Work out the finished part from the listing and answer in its coordinate system (mm). A direction names the side the tool comes from. Round coordinates to 2 decimals unless told otherwise and drop trailing zeros. Loops run counter-clockwise (first coordinate to the right, second up) from the corner with the lowest first, then second, coordinate; pieces in that order, holes last. Notation, with made-up numbers: (78, 29) -> (95, 29) arc R35 cw to (95, 67) -> close; hole circle Ø8 at (80.25, 32.25). An arc over 180 degrees is marked (long way). Use one line per item in the form item = value.
```python
from build123d import *

# Parameters (mm, degrees)
SKETCH_1_W                 = 410
SKETCH_1_H                 = 110
EXTRUDE_1_DEPTH            = 6
HOLE_WIZARD_3_AT_2_COUNT   = 2
HOLE_WIZARD_3_AT_2_PITCH   = 35
HOLE_WIZARD_3_AT_3_COUNT   = 2
HOLE_WIZARD_3_AT_3_PITCH   = 35
HOLE_WIZARD_3_AT_4_COUNT   = 2
HOLE_WIZARD_3_AT_4_PITCH   = 49.497474683
PATTERN_LINEAR_1_COUNT     = 2
PATTERN_LINEAR_1_PITCH     = 345
HOLE_WIZARD_2_D            = 9
HOLE_WIZARD_2_DEPTH        = 12.4
HOLE_WIZARD_2_CBORE_D      = 15
HOLE_WIZARD_2_CBORE_DEPTH  = 9
HOLE_WIZARD_2_TIP          = 2.703872786
HOLE_WIZARD_3_2_AT_2_COUNT = 2
HOLE_WIZARD_3_2_AT_2_PITCH = 40
SKETCH_14_R                = 4.5
CUT_EXTRUDE_1_DEPTH        = 213.588804973
CUT_EXTRUDE_2_DEPTH        = 9
PATTERN_LINEAR_2_COUNT     = 2
PATTERN_LINEAR_2_PITCH     = 350


with BuildPart() as part:
    # 草图1 → 凸台-拉伸1 (new, symmetric)
    with BuildSketch(Plane.XY):
        Rectangle(SKETCH_1_W, SKETCH_1_H)
    extrude(amount=EXTRUDE_1_DEPTH, both=True)

    # 草图3 → Hole Wizard 3 (revolve, cut)
    with BuildSketch(Plane(origin=(190, 30, -6), x_dir=(0, 1, 0), z_dir=(1, 0, 0))):
        Polygon((0, 0), (0, 14.382840043), (3.3, 12.4), (3.3, 6.8), (5.5, 6.8), (5.5, 0), align=None)
    hole_wizard_3 = revolve(axis=Axis((190, 30, -12.35), (0, 0, 1)), mode=Mode.SUBTRACT)

    # Hole Wizard 3 at 2: Hole Wizard 3 ×2
    with Locations(*[(-i * HOLE_WIZARD_3_AT_2_PITCH, 0, 0) for i in range(1, HOLE_WIZARD_3_AT_2_COUNT)]):
        add(hole_wizard_3, mode=Mode.SUBTRACT)

    # Hole Wizard 3 at 3: Hole Wizard 3 ×2
    with Locations(*[(0, -i * HOLE_WIZARD_3_AT_3_PITCH, 0) for i in range(1, HOLE_WIZARD_3_AT_3_COUNT)]):
        add(hole_wizard_3, mode=Mode.SUBTRACT)

    # Hole Wizard 3 at 4: Hole Wizard 3 ×2
    with Locations(*[Vector(-0.7071067811865477, -0.7071067811865474, 0) * (i * HOLE_WIZARD_3_AT_4_PITCH) for i in range(1, HOLE_WIZARD_3_AT_4_COUNT)]):
        add(hole_wizard_3, mode=Mode.SUBTRACT)

    # 阵列(线性)1: Hole Wizard 3 ×2
    with Locations(*[(-i * PATTERN_LINEAR_1_PITCH, 0, 0) for i in range(1, PATTERN_LINEAR_1_COUNT)]):
        add(hole_wizard_3, mode=Mode.SUBTRACT)

    # 阵列(线性)1 copy 1 sketch → 阵列(线性)1 copy 1 (revolve, cut)
    with BuildSketch(Plane(origin=(-190, 30, -6), x_dir=(0, 1, 0), z_dir=(1, 0, 0))):
        Polygon((0, 0), (0, 14.382840043), (3.3, 12.4), (3.3, 6.8), (5.5, 6.8), (5.5, 0), align=None)
    revolve(axis=Axis((-190, 30, -12.35), (0, 0, 1)), mode=Mode.SUBTRACT)

    # 阵列(线性)1 copy 2 sketch → 阵列(线性)1 copy 2 (revolve, cut)
    with BuildSketch(Plane(origin=(-155, -5, -6), x_dir=(0, 1, 0), z_dir=(1, 0, 0))):
        Polygon((0, 0), (0, 14.382840043), (3.3, 12.4), (3.3, 6.8), (5.5, 6.8), (5.5, 0), align=None)
    revolve(axis=Axis((-155, -5, -12.35), (0, 0, 1)), mode=Mode.SUBTRACT)

    # 阵列(线性)1 copy 3 sketch → 阵列(线性)1 copy 3 (revolve, cut)
    with BuildSketch(Plane(origin=(-190, -5, -6), x_dir=(0, 1, 0), z_dir=(1, 0, 0))):
        Polygon((0, 0), (0, 14.382840043), (3.3, 12.4), (3.3, 6.8), (5.5, 6.8), (5.5, 0), align=None)
    revolve(axis=Axis((-190, -5, -12.35), (0, 0, 1)), mode=Mode.SUBTRACT)

    # 打孔尺寸(%根据)内六角圆柱头螺钉的类型2
    with Locations(Plane(origin=(62.5, 25, -6), x_dir=(-1, 0, 0), z_dir=(0, 0, -1))):
        with Locations((0, 0), (0, -40), (65, -40), (65, 0)):
            CounterBoreHole(HOLE_WIZARD_2_D / 2, HOLE_WIZARD_2_CBORE_D / 2, HOLE_WIZARD_2_CBORE_DEPTH, depth=HOLE_WIZARD_2_DEPTH)
            with Locations((0, 0, -(HOLE_WIZARD_2_DEPTH + HOLE_WIZARD_2_TIP / 2))):  # 118° drill point
                Cone(0, HOLE_WIZARD_2_D / 2, HOLE_WIZARD_2_TIP, mode=Mode.SUBTRACT)

    # 草图5 → Hole Wizard 3 2 (revolve, cut)
    with BuildSketch(Plane(origin=(-175, 30, 6), x_dir=(0, -1, 0), z_dir=(1, 0, 0))):
        Polygon((0, 0), (0, 15.103872786), (4.5, 12.4), (4.5, 9), (7.5, 9), (7.5, 0), align=None)
    hole_wizard_3_2 = revolve(axis=Axis((-175, 30, 12.35), (0, 0, -1)), mode=Mode.SUBTRACT)

    # Hole Wizard 3 2 at 2: Hole Wizard 3 2 ×2
    with Locations(*[(0, -i * HOLE_WIZARD_3_2_AT_2_PITCH, 0) for i in range(1, HOLE_WIZARD_3_2_AT_2_COUNT)]):
        add(hole_wizard_3_2, mode=Mode.SUBTRACT)

    # 草图14 → 切除-拉伸1 (cut, through all)
    with BuildSketch(Plane.XY.offset(6)):
        with Locations((-175, 47.5)):
            Circle(SKETCH_14_R)
    cut_extrude_1 = extrude(amount=-CUT_EXTRUDE_1_DEPTH, mode=Mode.SUBTRACT)

    # 草图15 → 切除-拉伸2 (cut)
    with BuildSketch(Plane.XY.offset(6)):
        with BuildLine():
            Line((-182.5, 47.5), (-182.5, 101.28932806))
            ThreePointArc((-182.5, 101.28932806), (-175, 108.78932806), (-167.5, 101.28932806))
            Line((-167.5, 101.28932806), (-167.5, 47.5))
            ThreePointArc((-167.5, 47.5), (-175, 40), (-182.5, 47.5))
        make_face()
    cut_extrude_2 = extrude(amount=-CUT_EXTRUDE_2_DEPTH, mode=Mode.SUBTRACT)

    # 阵列(线性)2: Hole Wizard 3 2, 切除-拉伸1, 切除-拉伸2 ×2
    with Locations(*[(i * PATTERN_LINEAR_2_PITCH, 0, 0) for i in range(1, PATTERN_LINEAR_2_COUNT)]):
        add(hole_wizard_3_2, mode=Mode.SUBTRACT)
        add(cut_extrude_1, mode=Mode.SUBTRACT)
        add(cut_extrude_2, mode=Mode.SUBTRACT)

    # 阵列(线性)2 copy 1 sketch → 阵列(线性)2 copy 1 (revolve, cut)
    with BuildSketch(Plane(origin=(175, -10, 6), x_dir=(0, -1, 0), z_dir=(1, 0, 0))):
        Polygon((0, 0), (0, 15.103872786), (4.5, 12.4), (4.5, 9), (7.5, 9), (7.5, 0), align=None)
    revolve(axis=Axis((175, -10, 12.35), (0, 0, -1)), mode=Mode.SUBTRACT)


solid = part.part
```
(1) Find section A-A, the plane x = 175. Write down the section's boundary in (y, z).
Completed:
outline = (-55, -6) -> (-14.5, -6) -> (-14.5, -3) -> (-17.5, -3) -> (-17.5, 6) -> (-55, 6) -> close; (-5.5, -6) -> (25.5, -6) -> (25.5, -3) -> (22.5, -3) -> (22.5, 6) -> (-2.5, 6) -> (-2.5, -3) -> (-5.5, -3) -> close; (34.5, -6) -> (43, -6) -> (43, -3) -> (40, -3) -> (40, 6) -> (37.5, 6) -> (37.5, -3) -> (34.5, -3) -> close; (52, -6) -> (55, -6) -> (55, -3) -> (52, -3) -> close
(2) Find section B-B, the plane x = -2.5. Write down the section's boundary in (y, z).
Completed:
outline = (-55, -6) -> (-22.5, -6) -> (-22.5, 3) -> (-19.5, 3) -> (-19.5, 6) -> (-55, 6) -> close; (-10.5, 3) -> (-7.5, 3) -> (-7.5, -6) -> (17.5, -6) -> (17.5, 3) -> (20.5, 3) -> (20.5, 6) -> (-10.5, 6) -> close; (29.5, 3) -> (32.5, 3) -> (32.5, -6) -> (55, -6) -> (55, 6) -> (29.5, 6) -> close
(3) For faces 1 (the flat face through (-186, 30, 0.8)), 2 (the flat face through (-167.5, 51, 2)), 3 (the flat face through (180, -10, -3)), determine the directions among +Z, -Z, +X, -X, +Y, -Y from which every point of the face is accessible in a straight line to the end or side of a thin tool.
Completed:
face_1 = -Z
face_2 = +Z, +Y
face_3 = +Z
(4) Given P1, Ø7, axis at x = 175, y = 30, coming from the -Z side; P2, Ø16.5, axis at x = -175.5, y = 47, coming from the +Z side; P3, Ø10.5, axis at x = -175, y = 47.5, coming from the +Z side; P4, Ø8.5, axis at x = 190, y = -5, coming from the -Z side, each flat-ended and moving along its own axis, determine where each tip first touches the part or whether it passes through.
Completed:
P1 = through
P2 = 6
P3 = -3
P4 = 0.8
(5) Consider L1, parallel to Y at x = -190, z = -2.5; L2, parallel to Y at x = -175, z = 0.5; L3, parallel to X at y = -14.5, z = 0.5. Determine where each line is inside the solid, lowest interval first.
Completed:
L1 = -55 to -10.5, 0.5 to 24.5, 35.5 to 55
L2 = -55 to -17.5, -2.5 to 22.5, 37.5 to 40
L3 = -205 to -181, -169 to -9.98, 4.98 to 55.02, 69.98 to 169, 181 to 205
